```python
from build123d import *

# Parameters (mm, degrees)
SKETCH1_R           = 5.25
BOSS_EXTRUDE1_DEPTH = 3


with BuildPart() as part:
    # Sketch1 → Boss-Extrude1 (new, symmetric)
    with BuildSketch(Plane.XY):
        Polygon((-65, 15), (-60, 20), (60, 20), (65, 15), (65, -15), (60, -20), (-60, -20), (-65, -15), align=None)
        with Locations((-46, 0)):
            Circle(SKETCH1_R, mode=Mode.SUBTRACT)
        with Locations((46, 0)):
            Circle(SKETCH1_R, mode=Mode.SUBTRACT)
    extrude(amount=BOSS_EXTRUDE1_DEPTH, both=True)


solid = part.part
```
Check sheet for the modelled part. Datum: model origin and axes. Units: mm. Round coordinates to 2 decimals unless told otherwise and drop trailing zeros. Order: outer loops, then holes, each group sorted by start corner. A loop starts at its lowest first (then second) coordinate and runs counter-clockwise, first axis right, second up. Notation, with made-up numbers: (-27.75, 10.25) - (-21.75, 10.25) arc R8 cw to (-21.75, 20.25) - close; hole circle Ø2 at (5.25, 31.25). An arc over 180 degrees is marked (long way). Write item = value, one per line.
Q1. Section check B-B (z = -2.05). Record the boundary of the cut face in (x, y), and give its area (3 significant figures).
Computed:
outline = (-65, -15) - (-60, -20) - (60, -20) - (65, -15) - (65, 15) - (60, 20) - (-60, 20) - (-65, 15) - close; hole circle Ø10.5 at (-46, 0); hole circle Ø10.5 at (46, 0)
area = 4,980 mm^2
Q2. Section check D-D (x = -45). Record the boundary of the cut face in (y, z), and give its area (3 significant figures).
Computed:
outline = (-20, -3) - (-5.15, -3) - (-5.15, 3) - (-20, 3) - close; (5.15, -3) - (20, -3) - (20, 3) - (5.15, 3) - close
area = 178 mm^2
Q3. Draft check along Y on faces 1 (the face through (63, -17, 0)), 2 (the face through (-65, 0, 0)), 3 (the face through (-49.87, 3.55, -0.04)). Enter one of: pulls with the +Y half, pulls with the -Y half, needs draft (parallel to the pull), parting line crosses it, or undercut.
Computed:
face_1 = pulls with the -Y half
face_2 = needs draft
face_3 = undercut
Q4. Section check A-A (x = 46). Record the boundary of the cut face in (y, z).
Computed:
outline = (-20, -3) - (-5.25, -3) - (-5.25, 3) - (-20, 3) - close; (5.25, -3) - (20, -3) - (20, 3) - (5.25, 3) - close
Q5. Section check C-C (y = 3.5). Record the boundary of the cut face in (x, z).
Computed:
outline = (-65, -3) - (-49.91, -3) - (-49.91, 3) - (-65, 3) - close; (-42.09, -3) - (42.09, -3) - (42.09, 3) - (-42.09, 3) - close; (49.91, -3) - (65, -3) - (65, 3) - (49.91, 3) - close
Q6. Thickness scan on line 1 along Y through (x, z) = (46, -1.05); line 2 along X through (y, z) = (3, -0.25); line 3 along X through (y, z) = (-2.5, 2.5). Record the ranges inside material, lowest first.
Computed:
line_1 = -20 to -5.25, 5.25 to 20
line_2 = -65 to -50.31, -41.69 to 41.69, 50.31 to 65
line_3 = -65 to -50.62, -41.38 to 41.38, 50.62 to 65
